```python
from build123d import *

# Parameters (mm, degrees)
SKETCH1_W                = 37
SKETCH1_H                = 30
SKETCH1_W_2              = 20
SKETCH1_H_2              = 20
M4_CLEARANCE_HOLE1_D     = 4.5
M4_CLEARANCE_HOLE2_D     = 4.5
M4_CLEARANCE_HOLE2_DEPTH = 50
M4_CLEARANCE_HOLE2_TIP   = 1.351936393


with BuildPart() as part:
    # Sweep1: sweep along a path in Sketch2
    with BuildLine(Plane.XY) as sweep1_path:
        Line((0, 0), (175, 0))
        ThreePointArc((175, 0), (215, 40), (175, 80))
        Line((175, 80), (75, 80))
    # Sketch1 → Sweep1 (sweep)
    with BuildSketch(Plane(origin=(0, 0, 0), x_dir=(0, 0, -1), z_dir=(1, 0, 0))):
        Rectangle(SKETCH1_W, SKETCH1_H)
        Rectangle(SKETCH1_W_2, SKETCH1_H_2, mode=Mode.SUBTRACT)
    sweep(path=sweep1_path.line)

    # M4 Clearance Hole1 (through all)
    with Locations(Plane(origin=(0, 15, 0), x_dir=(1, 0, 0), z_dir=(0, 1, 0))):
        with Locations((8.5, 14.5), (8.5, -14.5)):
            Hole(M4_CLEARANCE_HOLE1_D / 2)

    # M4 Clearance Hole2
    with Locations(Plane(origin=(0, 95, 0), x_dir=(1, 0, 0), z_dir=(0, 1, 0))):
        with Locations((83.5, -14.5), (83.5, 14.5)):
            Hole(M4_CLEARANCE_HOLE2_D / 2, depth=M4_CLEARANCE_HOLE2_DEPTH)
            with Locations((0, 0, -(M4_CLEARANCE_HOLE2_DEPTH + M4_CLEARANCE_HOLE2_TIP / 2))):  # 118° drill point
                Cone(0, M4_CLEARANCE_HOLE2_D / 2, M4_CLEARANCE_HOLE2_TIP, mode=Mode.SUBTRACT)


solid = part.part
```
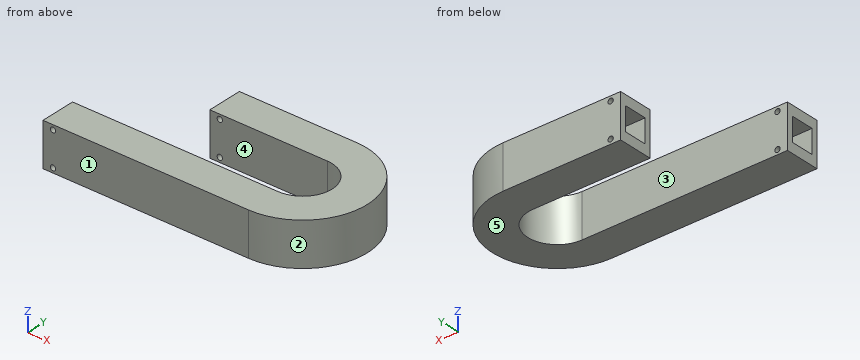
The model under review builds one solid part; all positions refer to its coordinate system, in mm. Face numbers are marked on the shaded views. A direction names the side the tool comes from. Give positions to 0.01 mm unless a question says otherwise; leave off trailing zeros. Write each loop counter-clockwise with the first axis right and the second up, starting at its lowest first coordinate (ties: lowest second). Pieces come first, ordered by that corner, then holes.
(1) The part is to be moulded in two halves that separate along Y. For the marked faces 1, 2 and 3, say which applies: released by +Y, released by -Y, zero draft, split by the parting line, or undercut.
(2) Tool access review of the marked faces 4 and 5: name each direction out of +Z, -Z, +X, -X, +Y, -Y from which nothing blocks a thin tool from reaching the whole face with its end or side.
(3) Consider section D-D, the plane y = 40. Give the boundary of the cut face in (x, z).
(4) Consider section B-B, the plane x = 83.5. Give the boundary of the cut face in (y, z).
(5) Consider section A-A, the plane x = 8.5. Give the boundary of the cut face in (y, z).
(6) To check wall thickness, follow L1, parallel to Z at x = 83.5, y = 88.25; L2, parallel to Y at x = 100, z = 6; L3, parallel to Z at x = 65.5, y = -3. State the ranges of each line that lie inside material, in increasing order.
(7) For P1, Ø3, axis at y = 62.5, z = -5.5, coming from the +X side; P2, Ø5, axis at x = 200, z = 5.5, coming from the -Y side; P3, Ø5, axis at x = 206, z = 6.5, coming from the -Y side; P4, Ø4, axis at x = 8.5, z = -14.5, coming from the +Y side, all flat-tipped, find the tip position at first contact; note any pin that passes through.
(8) Consider section C-C, the plane z = -14.5. Give the boundary of the cut face in (x, y).
Returned:
1. face 1: released by -Y
1. face 2: split by the parting line
1. face 3: undercut
2. face 4: +Z, -Z, -X
2. face 5: -Z, +X, -X, +Y, -Y
3. outline: (200, -18.5) - (230, -18.5) - (230, 18.5) - (200, 18.5) - close; hole (205, -10) - (225, -10) - (225, 10) - (205, 10) - close
4. outline: (-15, -18.5) - (15, -18.5) - (15, 18.5) - (-15, 18.5) - close; (65, -18.5) - (95, -18.5) - (95, -16.75) - (65, -16.75) - close; (65, -12.25) - (95, -12.25) - (95, 12.25) - (65, 12.25) - close; (65, 16.75) - (95, 16.75) - (95, 18.5) - (65, 18.5) - close; hole (-10, -10) - (10, -10) - (10, 10) - (-10, 10) - close; hole (70, -10) - (90, -10) - (90, 10) - (70, 10) - close
5. outline: (-15, -18.5) - (15, -18.5) - (15, -16.75) - (-15, -16.75) - close; (-15, -12.25) - (15, -12.25) - (15, 12.25) - (-15, 12.25) - close; (-15, 16.75) - (15, 16.75) - (15, 18.5) - (-15, 18.5) - close; hole (-10, -10) - (10, -10) - (10, 10) - (-10, 10) - close
6. L1: z = -18.5 to -16.75, -12.25 to -10, 10 to 12.25, 16.75 to 18.5
6. L2: y = -15 to -10, 10 to 15, 65 to 70, 90 to 95
6. L3: z = -18.5 to -10, 10 to 18.5
7. P1: stops at x = 225.83
7. P2: stops at y = -10.19
7. P3: stops at y = -7.04
7. P4: passes through
8. outline: (0, -15) - (6.25, -15) - (6.25, 15) - (0, 15) - close; (10.75, -15) - (175, -15) arc R55 ccw to (175, 95) - (85.75, 95) - (85.75, 65) - (175, 65) arc R25 cw to (175, 15) - (10.75, 15) - close; (75, 65) - (81.25, 65) - (81.25, 95) - (75, 95) - close
